Work out the finished part from the listing and answer in its coordinate system (mm). Face numbers are marked on the shaded views. A direction names the side the tool comes from. Round coordinates to 2 decimals unless told otherwise and drop trailing zeros. Loops run counter-clockwise (first coordinate to the right, second up) from the corner with the lowest first, then second, coordinate; pieces in that order, holes last. Notation, with made-up numbers: (87, 28) -> (104, 28) arc R20 ccw to (104, 36) -> close; hole circle Ø4 at (24.5, 34.25). An arc over 180 degrees is marked (long way). Write item = value, one per line. Start each with the question number.
```python
from build123d import *

# Parameters (mm, degrees)
SKETCH_1_W          = 120
SKETCH_1_H          = 120
EXTRUDE_1_DEPTH     = 15
SKETCH_3_R          = 90.791455295
SKETCH_3_R_2        = 60
CUT_EXTRUDE_1_DEPTH = 9
SKETCH_4_R          = 2.5
CUT_EXTRUDE_3_DEPTH = 91
FILLET_1_R          = 5
CUT_EXTRUDE_4_DEPTH = 91


with BuildPart() as part:
    # 草图1 → 凸台-拉伸1 (new, symmetric)
    with BuildSketch(Plane(origin=(0, 0, 0), x_dir=(1, 0, 0), z_dir=(0, 1, 0))):
        Rectangle(SKETCH_1_W, SKETCH_1_H)
    extrude(amount=EXTRUDE_1_DEPTH, both=True)

    # 草图3 → 切除-拉伸1 (cut, symmetric)
    with BuildSketch(Plane(origin=(0, 0, 0), x_dir=(1, 0, 0), z_dir=(0, 1, 0))):
        Circle(SKETCH_3_R)
        with Locations(Location((0, 0, 0), (0, 0, 270))):
            Circle(SKETCH_3_R_2, mode=Mode.SUBTRACT)
    extrude(amount=CUT_EXTRUDE_1_DEPTH, both=True, mode=Mode.SUBTRACT)

    # 草图4 → 切除-拉伸3 (cut, through all)
    with BuildSketch(Plane(origin=(0, 15, 0), x_dir=(1, 0, 0), z_dir=(0, 1, 0))):
        with Locations(Location((-52.5, 52.5, 0), (0, 0, 270))):
            Circle(SKETCH_4_R)
        with Locations(Location((-52.5, -52.5, 0), (0, 0, 270))):
            Circle(SKETCH_4_R)
        with Locations(Location((52.5, -52.5, 0), (0, 0, 270))):
            Circle(SKETCH_4_R)
        with Locations(Location((52.5, 52.5, 0), (0, 0, 270))):
            Circle(SKETCH_4_R)
    extrude(amount=-CUT_EXTRUDE_3_DEPTH, mode=Mode.SUBTRACT)

    # 圆角1
    fillet_1_edges = [part.edges().sort_by_distance(p)[0] for p in [
        (60, -12, 60),
        (-60, -12, 60),
        (-60, -12, -60),
        (60, -12, -60),
        (60, 12, 60),
        (-60, 12, 60),
        (-60, 12, -60),
        (60, 12, -60),
    ]]
    fillet(fillet_1_edges, radius=FILLET_1_R)

    # 草图5 → 切除-拉伸4 (cut, through all)
    with BuildSketch(Plane(origin=(0, 15, 0), x_dir=(1, 0, 0), z_dir=(0, 1, 0))):
        with BuildLine():
            ThreePointArc((-9.659258263, 2.588190451), (-7.071067812, 7.071067812), (-2.588190451, 9.659258263))
            Line((-2.588190451, 9.659258263), (-14.235047481, 53.125920446))
            ThreePointArc((-14.235047481, 53.125920446), (-38.890872965, 38.890872965), (-53.125920446, 14.235047481))
            Line((-53.125920446, 14.235047481), (-9.659258263, 2.588190451))
        make_face()
        with BuildLine():
            Line((14.235047481, 53.125920446), (2.588190451, 9.659258263))
            ThreePointArc((2.588190451, 9.659258263), (7.071067812, 7.071067812), (9.659258263, 2.588190451))
            Line((9.659258263, 2.588190451), (53.125920446, 14.235047481))
            ThreePointArc((53.125920446, 14.235047481), (38.890872965, 38.890872965), (14.235047481, 53.125920446))
        make_face()
        with BuildLine():
            ThreePointArc((9.659258263, -2.588190451), (7.071067812, -7.071067812), (2.588190451, -9.659258263))
            Line((2.588190451, -9.659258263), (14.235047481, -53.125920446))
            ThreePointArc((14.235047481, -53.125920446), (38.890872965, -38.890872965), (53.125920446, -14.235047481))
            Line((53.125920446, -14.235047481), (9.659258263, -2.588190451))
        make_face()
        with BuildLine():
            Line((-14.235047481, -53.125920446), (-2.588190451, -9.659258263))
            ThreePointArc((-2.588190451, -9.659258263), (-7.071067812, -7.071067812), (-9.659258263, -2.588190451))
            Line((-9.659258263, -2.588190451), (-53.125920446, -14.235047481))
            ThreePointArc((-53.125920446, -14.235047481), (-38.890872965, -38.890872965), (-14.235047481, -53.125920446))
        make_face()
    extrude(amount=-CUT_EXTRUDE_4_DEPTH, mode=Mode.SUBTRACT)


solid = part.part
```
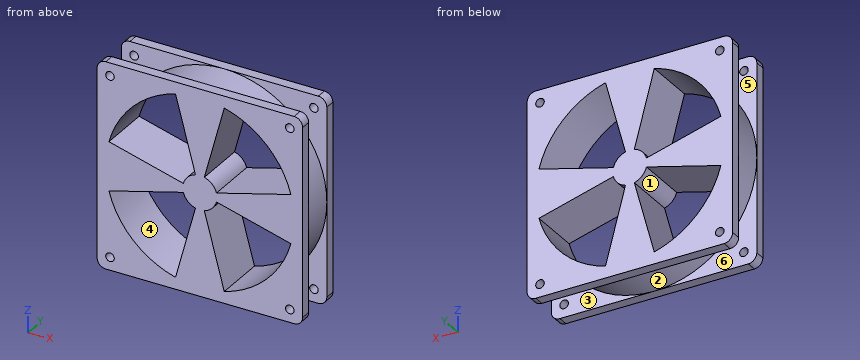
Item 1: Section A-A (y = 6.25) is taken. Determine the outline of the cut face in (x, z), then the cut area to 3 significant figures.
Item 2: The mould has two halves that part along X. Classify the marked faces 1, 2 and 3: pulls with the +X half, pulls with the -X half, needs draft (parallel to the pull), parting line crosses it, or undercut.
Item 3: Flat-ended cylindrical pins translate along their axes: pin 1 (6 mm diameter, centred on x = 13, y = 0.5, fed in from +Z); pin 2 (5 mm diameter, centred on x = 21.5, y = 4.5, fed in from -Z); pin 3 (6 mm diameter, centred on x = -9, y = -2.5, fed in from -Z). Find the tip coordinate at first contact, or state that the pin passes through.
Item 4: A tool of negligible diameter and unlimited length cuts with its end or side. For the marked faces 4, 5 and 6, from which of +Z, -Z, +X, -X, +Y, -Y can it reach the whole face along a straight path? Write none if from no direction.
Item 5: Section B-B (x = -24) is taken. Determine the outline of the cut face in (y, z).
Item 6: Section C-C (z = 45) is taken. Determine the outline of the cut face in (x, y).
Item 7: Find the intervals of material crossed by line 1 along Z through (x, y) = (-34, -2.75); line 2 along X through (y, z) = (3.5, 18); line 3 along Z through (x, y) = (22, 0), in increasing order. Write a range as [from, to].
Worked answers:
q1.outline = circle Ø120 at (0, 0); hole (-53.13, -14.24) arc R55 ccw to (-14.24, -53.13) -> (-2.59, -9.66) arc R10 cw to (-9.66, -2.59) -> close; hole (-53.13, 14.24) -> (-9.66, 2.59) arc R10 cw to (-2.59, 9.66) -> (-14.24, 53.13) arc R55 ccw to start; hole (2.59, -9.66) -> (14.24, -53.13) arc R55 ccw to (53.13, -14.24) -> (9.66, -2.59) arc R10 cw to start; hole (2.59, 9.66) arc R10 cw to (9.66, 2.59) -> (53.13, 14.24) arc R55 ccw to (14.24, 53.13) -> close
q1.area = 5,180 mm2
q2.face_1 = undercut
q2.face_2 = parting line crosses it
q2.face_3 = needs draft
q3.pin_1 = 59.16
q3.pin_2 = -56.91
q3.pin_3 = -59.7
q4.face_4 = +Y, -Y
q4.face_5 = +Z, -X
q4.face_6 = -Z, -X
q5.outline = (-15, -60) -> (-9, -60) -> (-9, -54.99) -> (9, -54.99) -> (9, -60) -> (15, -60) -> (15, -49.49) -> (-15, -49.49) -> close; (-15, -6.43) -> (15, -6.43) -> (15, 6.43) -> (-15, 6.43) -> close; (-15, 49.49) -> (15, 49.49) -> (15, 60) -> (9, 60) -> (9, 54.99) -> (-9, 54.99) -> (-9, 60) -> (-15, 60) -> close
q6.outline = (-60, -15) -> (-31.62, -15) -> (-31.62, 15) -> (-60, 15) -> (-60, 9) -> (-39.69, 9) -> (-39.69, -9) -> (-60, -9) -> close; (-12.06, -15) -> (12.06, -15) -> (12.06, 15) -> (-12.06, 15) -> close; (31.62, -15) -> (60, -15) -> (60, -9) -> (39.69, -9) -> (39.69, 9) -> (60, 9) -> (60, 15) -> (31.62, 15) -> close
q7.line_1 = [-49.44, -43.23], [-9.11, 9.11], [43.23, 49.44]
q7.line_2 = [-57.24, -51.97], [-4.82, 4.82], [51.97, 57.24]
q7.line_3 = [-55.82, -50.41], [-5.89, 5.89], [50.41, 55.82]
